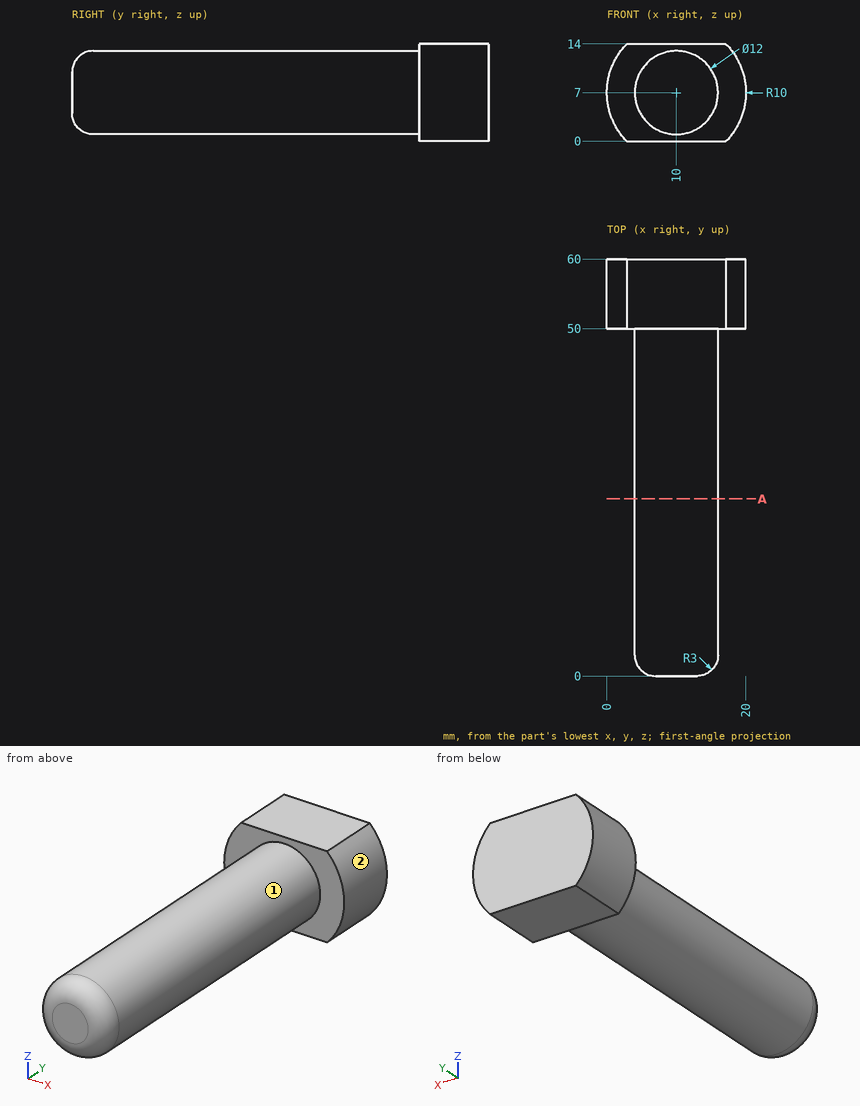
Geometry: see drawing. Coordinates: mm, zero at the bounding-box minimum. A direction names the side the tool comes from. Give positions to 0.01 mm unless a question says otherwise; leave off trailing zeros. Order: outer loops, then holes, each group sorted by start corner. A loop starts at its lowest first (then second) coordinate and runs counter-clockwise, first axis right, second up.
Q1. Ray query, probe 1 along Y at (x, z) = (1, 8); probe 2 along X at (y, z) = (46, 4.5); probe 3 along Z at (x, y) = (5.25, 40.5). Return the intervals inside material, ascending.
Checked values:
probe 1: y = 50 to 60
probe 2: x = 4.55 to 15.45
probe 3: z = 3.33 to 10.67
Q2. Contact query for flat-ended pins moving along their axis: pin 1 Ø1 at (x, y) = (15, 37) entering from -Z; pin 2 Ø1 at (y, z) = (39.5, 8) entering from +X; pin 3 Ø6 at (x, y) = (9.5, 42.5) entering from +Z. Output: stop coordinate, or through.
Checked values:
pin 1: stops at z = 3.03
pin 2: stops at x = 15.98
pin 3: stops at z = 13
Q3. Section A-A on y = 25.5. Output: boundary loops of the cut face in (x, z).
Checked values:
outline: circle Ø12 at (10, 7)
Q4. Set-up query: the marked faces 1 and 2. Return all of +Z, -Z, +X, -X, +Y, -Y with unobstructed straight access to the full face (end or side cutting, diameter ignored); none if empty.
Checked values:
face 1: -Y
face 2: +X, +Y, -Y
